```python
from build123d import *

# Parameters (mm, degrees)
BOSS_EXTRUDE1_START     = 100
SKETCH1_R               = 80
SKETCH1_R_2             = 50
BOSS_EXTRUDE1_DEPTH     = 900
BOSS_EXTRUDE2_DEPTH     = 400
CUT_EXTRUDE2_DEPTH      = 1417.518619715
CUT_EXTRUDE2_DEPTH_BACK = 1417.518619715
CUT_EXTRUDE3_DEPTH      = 1417.518619715
CUT_EXTRUDE3_DEPTH_BACK = 1417.518619715
SKETCH_4_5_2_R          = 50


with BuildPart() as part:
    # Sketch1 → Boss-Extrude1 (new body)
    with BuildSketch(Plane(origin=(0, 0, 0), x_dir=(0, 0, -1), z_dir=(1, 0, 0)).offset(BOSS_EXTRUDE1_START)):
        Circle(SKETCH1_R)
        Circle(SKETCH1_R_2, mode=Mode.SUBTRACT)
    extrude(amount=BOSS_EXTRUDE1_DEPTH)

    # Sketch3 → Boss-Extrude2 (add)
    with BuildSketch(Plane(origin=(1000, 0, 0), x_dir=(0, 0, -1), z_dir=(1, 0, 0))):
        with BuildLine():
            Line((-75, 129.903810568), (-75, -129.903810568))
            ThreePointArc((-75, -129.903810568), (0, -150), (75, -129.903810568))
            Line((75, -129.903810568), (75, 129.903810568))
            ThreePointArc((75, 129.903810568), (0, 150), (-75, 129.903810568))
        make_face()
    extrude(amount=BOSS_EXTRUDE2_DEPTH)

    # Sketch 4_5 → Cut-Extrude2 (cut, two sides: drawn at the far end of the back side and taken through both)
    with BuildSketch(Plane.XY.offset(75).offset(-CUT_EXTRUDE2_DEPTH_BACK)):
        with BuildLine():
            Line((1250, 150), (1455.357524725, 150))
            Line((1455.357524725, 150), (1455.357524725, -150))
            Line((1455.357524725, -150), (1250, -150))
            ThreePointArc((1250, -150), (1400, 0), (1250, 150))
        make_face()
    extrude(amount=CUT_EXTRUDE2_DEPTH + CUT_EXTRUDE2_DEPTH_BACK, mode=Mode.SUBTRACT)

    # Sketch 4_5 2 → Cut-Extrude3 (cut, two sides: drawn at the far end of the back side and taken through both)
    with BuildSketch(Plane.XY.offset(75).offset(-CUT_EXTRUDE3_DEPTH_BACK)):
        with Locations((1250, 0)):
            Circle(SKETCH_4_5_2_R)
    extrude(amount=CUT_EXTRUDE3_DEPTH + CUT_EXTRUDE3_DEPTH_BACK, mode=Mode.SUBTRACT)


solid = part.part
```
Check sheet for the modelled part. Datum: model origin and axes. Units: mm. A direction names the side the tool comes from. Round coordinates to 2 decimals unless told otherwise and drop trailing zeros. Order: outer loops, then holes, each group sorted by start corner. A loop starts at its lowest first (then second) coordinate and runs counter-clockwise, first axis right, second up. Notation, with made-up numbers: (-31.5, 52) - (-23.5, 52) arc R21 cw to (-23.5, 69) - close; hole circle Ø10 at (88, 34). An arc over 180 degrees is marked (long way). Write item = value, one per line.
Q1. Thickness scan on line 1 along Y through (x, z) = (300, 0); line 2 along X through (y, z) = (-1, 63.5); line 3 along X through (y, z) = (130, 34). Record the ranges inside material, lowest first.
Computed:
line_1 = -80 to -50, 50 to 80
line_2 = 100 to 1200.01, 1299.99 to 1400
line_3 = 1000 to 1324.83
Q2. Section check A-A (y = 0). Record the boundary of the cut face in (x, z), and give its area (3 significant figures).
Computed:
outline = (100, -80) - (1000, -80) - (1000, -75) - (1200, -75) - (1200, 75) - (1000, 75) - (1000, 80) - (100, 80) - (100, 50) - (1000, 50) - (1000, -50) - (100, -50) - close; (1300, -75) - (1400, -75) - (1400, 75) - (1300, 75) - close
area = 99,000 mm^2
Q3. Section check D-D (y = -66.5). Record the boundary of the cut face in (x, z), and give its area (3 significant figures).
Computed:
outline = (100, -44.47) - (1000, -44.47) - (1000, -75) - (1384.45, -75) - (1384.45, 75) - (1000, 75) - (1000, 44.47) - (100, 44.47) - close
area = 138,000 mm^2
Q4. Go/stop test with flat-tipped pins: pin 1 (4 mm diameter, centred on y = 21.5, z = 7.5, fed in from -X); pin 2 (5 mm diameter, centred on y = -69.5, z = -30, fed in from +X); pin 3 (5.5 mm diameter, centred on y = -13.5, z = 78, fed in from +X). Record where each tip stops, or that it passes through.
Computed:
pin_1 = 1000
pin_2 = 1384.21
pin_3 = 1000
Q5. Section check C-C (x = 647.5). Record the boundary of the cut face in (y, z).
Computed:
outline = circle Ø160 at (0, 0); hole circle Ø100 at (0, 0)
Q6. Draft check along Z on faces 1 (the face through (1000, 1, 1)), 2 (the face through (543.7, -78.1, 17.34)), 3 (the face through (1197, 2, 75)). Enter one of: pulls with the +Z half, pulls with the -Z half, needs draft (parallel to the pull), parting line crosses it, or undercut.
Computed:
face_1 = undercut
face_2 = parting line crosses it
face_3 = pulls with the +Z half
Q7. Section check B-B (z = 0). Record the boundary of the cut face in (x, y).
Computed:
outline = (100, -80) - (1000, -80) - (1000, -150) - (1250, -150) arc R150 ccw to (1250, 150) - (1000, 150) - (1000, 80) - (100, 80) - (100, 50) - (1000, 50) - (1000, -50) - (100, -50) - close; hole circle Ø100 at (1250, 0)
Q8. Tool access check on faces 4 (the face through (1197, -2, -75)), 5 (the face through (543.7, 15.02, -47.69)), 6 (the face through (1124.114, 149.996, -1.1)). Record the directions out of +Z, -Z, +X, -X, +Y, -Y that give a thin tool (end or side, any length) a straight path to the whole face; none if there is none.
Computed:
face_4 = -Z, +X, +Y, -Y
face_5 = -X
face_6 = +X, -X, +Y
